Part model, mm, in its own coordinate system. A direction names the side the tool comes from. Round coordinates to 2 decimals unless told otherwise and drop trailing zeros. Loops run counter-clockwise (first coordinate to the right, second up) from the corner with the lowest first, then second, coordinate; pieces in that order, holes last. Notation, with made-up numbers: (46.25, 42) - (77.25, 42) arc R28 ccw to (77.25, 68) - close; hole circle Ø10 at (72, 12). An arc over 180 degrees is marked (long way). Put each result on its own line as item: value.
from build123d import *

# Parameters (mm, degrees)
RING_BODY_DEPTH       = 4.5
EDGE_CHAMFER_1MM_SIZE = 1
RADIAL_CUT_DEPTH      = 38.7458607
RADIAL_CUT_DEPTH_BACK = 38.7458607
RADIAL_CUT_SKETCH_R   = 2
SLOT_START            = 7
SLOT_SKETCH_R         = 3
SLOT_CUT_DEPTH        = 25


with BuildPart() as part:
    # Ring Profile Sketch → Ring Body (new, symmetric)
    with BuildSketch(Plane.XY):
        with BuildLine():
            Line((-0.75, 17.483921185), (-0.75, 21.843890817))
            Line((-0.75, 21.843890817), (0.75, 21.843890817))
            Line((0.75, 21.843890817), (0.75, 17.483921185))
            ThreePointArc((0.75, 17.483921185), (17.5, 0), (0.75, -17.483921185))
            Line((0.75, -17.483921185), (0.75, -26.489384666))
            ThreePointArc((0.75, -26.489384666), (0, 26.5), (-0.75, -26.489384666))
            Line((-0.75, -26.489384666), (-0.75, -17.483921185))
            ThreePointArc((-0.75, -17.483921185), (-17.5, 0), (-0.75, 17.483921185))
        make_face()
    extrude(amount=RING_BODY_DEPTH, both=True)

    # Edge Chamfer 1mm
    edge_chamfer_1mm_edges = [part.edges().sort_by_distance(p)[0] for p in [
        (-17.5, 0, -4.5),
        (17.5, 0, 4.5),
        (0, 26.5, 4.5),
        (-17.5, 0, 4.5),
        (0, 26.5, -4.5),
        (17.5, 0, -4.5),
    ]]
    chamfer(edge_chamfer_1mm_edges, length=EDGE_CHAMFER_1MM_SIZE)

    # Radial Cut Sketch → Radial Cut (cut, two sides: drawn at the far end of the back side and taken through both)
    with BuildSketch(Plane(origin=(0, 0, 0), x_dir=(0, 0, -1), z_dir=(1, 0, 0)).offset(-RADIAL_CUT_DEPTH_BACK)):
        with Locations((0, -21.983921185)):
            Circle(RADIAL_CUT_SKETCH_R)
    extrude(amount=RADIAL_CUT_DEPTH + RADIAL_CUT_DEPTH_BACK, mode=Mode.SUBTRACT)

    # Slot Sketch → Slot Cut (cut)
    with BuildSketch(Plane(origin=(0, 0, 0), x_dir=(0, 0, -1), z_dir=(1, 0, 0)).offset(SLOT_START)):
        with Locations(Location((0, -21.983921185, 0), (0, 0, 180))):
            Circle(SLOT_SKETCH_R)
    slot_cut = extrude(amount=SLOT_CUT_DEPTH, mode=Mode.SUBTRACT)

    # Slot Mirror: Slot Cut across plane
    add(slot_cut.mirror(Plane(origin=(0, 0, 0), x_dir=(0, 0, 1), z_dir=(1, 0, 0))), mode=Mode.SUBTRACT)


solid = part.part
1. Tool access for faces 4 (the flat face through (-0.75, 20, 0)), 5 (the conical face through (18, 0, 4)), 6 (the conical face through (-18, 0, -4)), 7 (the cylindrical face through (17.496, 0.374, 0.049)), 8 (the cylindrical face through (11.388, -19.055, -0.65)): list every direction of +Z, -Z, +X, -X, +Y, -Y with a clear straight run to the whole face (end or side of a thin tool).
A:
face 4: +Z, -Z, -Y
face 5: +Z
face 6: -Z
face 7: +Z, -Z
face 8: +X
2. Band-saw the part on C-C (x = 0). List the corners of the cut face in (y, z), plus the area to 3 significant figures.
A:
outline: (21.84, -4.5) - (25.5, -4.5) - (26.5, -3.5) - (26.5, 3.5) - (25.5, 4.5) - (21.84, 4.5) - close
area: 40.9 mm²
3. Pin check, flat tips, straight feed: P1, Ø5, axis at y = -4.5, z = 2, coming from the -X side; P2, Ø1.5, axis at x = -5, z = -3, coming from the -Y side; P3, Ø5, axis at y = 20.5, z = 0.5, coming from the +X side; P4, Ø3.5, axis at y = -21.98, z = 0, coming from the +X side. Stop position of each tip, or through.
A:
P1: stops at x = -26.42
P2: stops at y = -26.16
P3: stops at x = 19.45
P4: passes through
4. Band-saw the part on A-A (y = 0). List the corners of the cut face in (x, z), plus the area to 3 significant figures.
A:
outline: (-26.5, -3.5) - (-25.5, -4.5) - (-18.5, -4.5) - (-17.5, -3.5) - (-17.5, 3.5) - (-18.5, 4.5) - (-25.5, 4.5) - (-26.5, 3.5) - close; (17.5, -3.5) - (18.5, -4.5) - (25.5, -4.5) - (26.5, -3.5) - (26.5, 3.5) - (25.5, 4.5) - (18.5, 4.5) - (17.5, 3.5) - close
area: 158 mm²
5. Band-saw the part on B-B (z = 0). List the corners of the cut face in (x, y).
A:
outline: (-18.49, -18.98) - (-7, -18.98) - (-7, -19.98) - (-0.75, -19.98) - (-0.75, -17.48) arc R17.5 cw to (-0.75, 17.48) - (-0.75, 21.84) - (0.75, 21.84) - (0.75, 17.48) arc R17.5 cw to (0.75, -17.48) - (0.75, -19.98) - (7, -19.98) - (7, -18.98) - (18.49, -18.98) arc R26.5 ccw (long way) to start; (-8.83, -24.98) arc R26.5 ccw to (-0.75, -26.49) - (-0.75, -23.98) - (-7, -23.98) - (-7, -24.98) - close; (0.75, -26.49) arc R26.5 ccw to (8.83, -24.98) - (7, -24.98) - (7, -23.98) - (0.75, -23.98) - close
6. Two-plate mould, pull along Y, no slides. Class faces 1 (the cylindrical face through (-3.919, -23.936, 0.434)), 2 (the flat face through (0.75, -24, 1)), 3 (the conical face through (1.118, 25.635, 4.34)): pulls with the +Y half, pulls with the -Y half, needs draft (parallel to the pull), parting line crosses it, or undercut.
A:
face 1: undercut
face 2: needs draft
face 3: parting line crosses it
7. Probe line 1 along Y through (x, z) = (3, -1); line 2 along X through (y, z) = (19, 3.5); line 3 along Y through (x, z) = (3, 0). List the from-to ranges inside material, lowest first. Write a range as [from, to].
A:
line 1: y = [-26.33, -23.72], [-20.25, -17.24], [17.24, 26.33]
line 2: x = [-18.47, -0.75], [0.75, 18.47]
line 3: y = [-26.33, -23.98], [-19.98, -17.24], [17.24, 26.33]
